Part model, mm, in its own coordinate system. Face numbers are marked on the shaded views. A direction names the side the tool comes from. Give positions to 0.01 mm unless a question says otherwise; leave off trailing zeros. Order: outer loops, then holes, each group sorted by start corner. A loop starts at its lowest first (then second) coordinate and runs counter-clockwise, first axis right, second up. Notation, with made-up numbers: (85, 39) - (93, 39) arc R26 ccw to (93, 74) - close; hole circle Ø3 at (63, 53.25). An arc over 180 degrees is marked (long way). One line per item, written item: value.
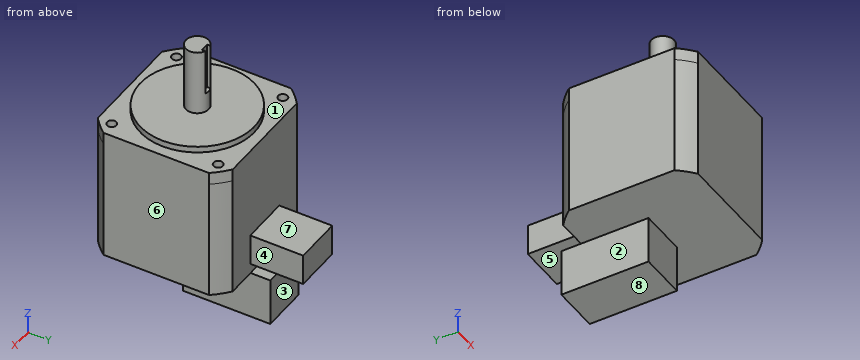
```python
from build123d import *
from build123d.topology import SkipClean

# Parameters (mm, degrees)
SKETCH1_W           = 130
SKETCH1_H           = 130
BOSS_EXTRUDE1_DEPTH = 12
SKETCH2_R           = 55
BOSS_EXTRUDE2_DEPTH = 6
SKETCH3_R           = 11
BOSS_EXTRUDE3_DEPTH = 64
SKETCH4_OUTSIDE_W   = 172.262
SKETCH4_OUTSIDE_H   = 172.262
SKETCH4_OUTSIDE_R   = 82.5
CUT_EXTRUDE1_DEPTH  = 64
CIRPATTERN1_COUNT   = 4
BOSS_EXTRUDE4_DEPTH = 117
SKETCH8_W           = 45
SKETCH8_H           = 84
BOSS_EXTRUDE5_DEPTH = 46
SKETCH9_W           = 30
SKETCH9_H           = 51
BOSS_EXTRUDE6_DEPTH = 23
SKETCH10_W          = 8
SKETCH10_H          = 10
CUT_EXTRUDE2_DEPTH  = 45


with BuildPart() as part:
    # Sketch1 → Boss-Extrude1 (new body)
    with BuildSketch(Plane.XY):
        Rectangle(SKETCH1_W, SKETCH1_H)
    extrude(amount=BOSS_EXTRUDE1_DEPTH)

    # Sketch2 → Boss-Extrude2 (add)
    with BuildSketch(Plane.XY.offset(12)):
        Circle(SKETCH2_R)
    extrude(amount=BOSS_EXTRUDE2_DEPTH)

    # Sketch3 → Boss-Extrude3 (add)
    with BuildSketch(Plane.XY.offset(18)):
        Circle(SKETCH3_R)
    extrude(amount=BOSS_EXTRUDE3_DEPTH)

    # Sketch4 outside → Cut-Extrude1 (cut)
    with BuildSketch(Plane.XY.offset(12)):
        Rectangle(SKETCH4_OUTSIDE_W, SKETCH4_OUTSIDE_H)
        Circle(SKETCH4_OUTSIDE_R, mode=Mode.SUBTRACT)
    extrude(amount=-CUT_EXTRUDE1_DEPTH, mode=Mode.SUBTRACT)

    # Sketch5 → Ø9.0 (9) Diameter Hole1 (revolve, cut)
    with BuildSketch(Plane(origin=(-51.265241636, 51.265241636, 12), x_dir=(0, -1, 0), z_dir=(1, 0, 0))):
        Polygon((0, 0), (0, 402.703872786), (4.5, 400), (4.5, 0), align=None)
    f_9_0_9_diameter_hole1 = revolve(axis=Axis((-51.265241636, 51.265241636, 18.35), (0, 0, -1)), mode=Mode.SUBTRACT)

    # CirPattern1: Ø9.0 (9) Diameter Hole1 ×4 about axis
    cirpattern1_axis = Axis((0, 0, 0), (0, 0, 1))
    for i in range(1, CIRPATTERN1_COUNT):
        add(f_9_0_9_diameter_hole1.rotate(cirpattern1_axis, i * 360 / CIRPATTERN1_COUNT), mode=Mode.SUBTRACT)

    # Sketch7 → Boss-Extrude4 (add)
    with SkipClean():  # the faces are left unmerged after this step: merging them gives an invalid solid
        with BuildSketch(Plane(origin=(0, 0, 0), x_dir=(-1, 0, 0), z_dir=(0, 0, -1))):
            with BuildLine():
                Line((-65, 50.806003582), (-65, -50.806003582))
                ThreePointArc((-65, -50.806003582), (-58.336309448, -58.336309448), (-50.806003582, -65))
                Line((-50.806003582, -65), (50.806003582, -65))
                ThreePointArc((50.806003582, -65), (58.336309448, -58.336309448), (65, -50.806003582))
                Line((65, -50.806003582), (65, 50.806003582))
                ThreePointArc((65, 50.806003582), (58.336309448, 58.336309448), (50.806003582, 65))
                Line((50.806003582, 65), (-50.806003582, 65))
                ThreePointArc((-50.806003582, 65), (-58.336309448, 58.336309448), (-65, 50.806003582))
            make_face()
        extrude(amount=BOSS_EXTRUDE4_DEPTH)

    # Sketch8 → Boss-Extrude5 (add)
    with SkipClean():  # the faces are left unmerged after this step: merging them gives an invalid solid
        with BuildSketch(Plane(origin=(0, 0, -117), x_dir=(-1, 0, 0), z_dir=(0, 0, -1))):
            with Locations((0, 42)):
                Rectangle(SKETCH8_W, SKETCH8_H)
        extrude(amount=BOSS_EXTRUDE5_DEPTH)

    # Sketch9 → Boss-Extrude6 (add, symmetric)
    with SkipClean():  # the faces are left unmerged after this step: merging them gives an invalid solid
        with BuildSketch(Plane(origin=(0, 0, 0), x_dir=(0, 0, -1), z_dir=(1, 0, 0))):
            with Locations((92, 90.5)):
                Rectangle(SKETCH9_W, SKETCH9_H)
        extrude(amount=BOSS_EXTRUDE6_DEPTH, both=True)

    # Sketch10 → Cut-Extrude2 (cut)
    with SkipClean():  # the faces are left unmerged after this step: merging them gives an invalid solid
        with BuildSketch(Plane.XY.offset(82)):
            with Locations((0, 12)):
                Rectangle(SKETCH10_W, SKETCH10_H)
        extrude(amount=-CUT_EXTRUDE2_DEPTH, mode=Mode.SUBTRACT)


solid = part.part
```
1) Two-plate mould, pull along Z, no slides. Class the marked faces 5, 6, 7 and 8: pulls with the +Z half, pulls with the -Z half, needs draft (parallel to the pull), parting line crosses it, or undercut.
Answer:
face 5: undercut
face 6: needs draft
face 7: pulls with the +Z half
face 8: pulls with the -Z half
2) Wall check: line 1 along Z through (x, y) = (19.5, -2); line 2 along Y through (x, z) = (-0.5, -61.5); line 3 along Z through (x, y) = (-44.5, 37.5). Give the ranges that are in metal, low to high. Write a range as [from, to].
Answer:
line 1: z = [-117, 18]
line 2: y = [-65, 65]
line 3: z = [-117, 12]
3) Slice it at B-B on z = -67. Write the cut outline in (x, y), then the cut area to 3 significant figures.
Answer:
outline: (-65, -50.81) arc R82.5 ccw to (-50.81, -65) - (50.81, -65) arc R82.5 ccw to (65, -50.81) - (65, 50.81) arc R82.5 ccw to (50.81, 65) - (-50.81, 65) arc R82.5 ccw to (-65, 50.81) - close
area: 16,500 mm2
4) Drop flat-ended pins along their axis: P1, Ø10.5, axis at x = -51.27, y = 51.27, coming from the -Z side; P2, Ø4, axis at x = 1.5, z = 57, coming from the +Y side; P3, Ø10, axis at x = 45.5, z = -14, coming from the +Y side. Give the stop position or say it passes through.
Answer:
P1: stops at z = -117
P2: stops at y = 7
P3: stops at y = 65
5) Slice it at C-C on y = 33.5. Write the cut outline in (x, z), then the cut area to 3 significant figures.
Answer:
outline: (-65, -117) - (-22.5, -117) - (-22.5, -163) - (22.5, -163) - (22.5, -117) - (65, -117) - (65, 12) - (43.62, 12) - (43.62, 18) - (-43.62, 18) - (-43.62, 12) - (-65, 12) - close
area: 19,400 mm2
6) Which spindle directions (+Z, -Z, +X, -X, +Y, -Y) get a long thin tool onto all of the face, cutting with end or side? Do the marked faces 1, 2, 3 and 4. Say none if no direction does.
Answer:
face 1: +Z
face 2: -Z, -X, +Y, -Y
face 3: -Z, +X, -X, +Y
face 4: +Z, -Z, +X, +Y
7) Slice it at A-A on x = 0. Write the cut outline in (y, z).
Answer:
outline: (-65, -117) - (0, -117) - (0, -163) - (84, -163) - (84, -117) - (65, -117) - (65, -107) - (116, -107) - (116, -77) - (65, -77) - (65, 12) - (55, 12) - (55, 18) - (11, 18) - (11, 37) - (7, 37) - (7, 82) - (-11, 82) - (-11, 18) - (-55, 18) - (-55, 12) - (-65, 12) - close
8) Slice it at D-D on z = -120.5. Write the cut outline in (x, y), then the cut area to 3 significant figures.
Answer:
outline: (-22.5, 0) - (22.5, 0) - (22.5, 84) - (-22.5, 84) - close
area: 3,780 mm2
